from build123d import *

# Parameters (mm, degrees)
BASE_PLATE_SKETCH_R    = 15
BASE_PLATE_DEPTH       = 10
CENTRE_COLUMN_SKETCH_R = 15
CENTRE_COLUMN_DEPTH    = 50
TOP_PLATE_SKETCH_R     = 15
TOP_PLATE_DEPTH        = 10
OCTAGON_BOSS_SKETCH_R  = 25
OCTAGON_BOSS_DEPTH     = 10
CROSS_HOLE_18_D        = 18


with BuildPart() as part:
    # Base Plate Sketch → Base Plate (new body)
    with BuildSketch(Plane(origin=(0, 0, 0), x_dir=(1, 0, 0), z_dir=(0, 1, 0))):
        with BuildLine():
            Line((-40, 50), (40, 50))
            ThreePointArc((40, 50), (47.071067812, 47.071067812), (50, 40))
            Line((50, 40), (50, -40))
            ThreePointArc((50, -40), (47.071067812, -47.071067812), (40, -50))
            Line((40, -50), (-40, -50))
            ThreePointArc((-40, -50), (-47.071067812, -47.071067812), (-50, -40))
            Line((-50, -40), (-50, 40))
            ThreePointArc((-50, 40), (-47.071067812, 47.071067812), (-40, 50))
        make_face()
        with Locations(Location((0, 0, 0), (0, 0, 270))):
            Circle(BASE_PLATE_SKETCH_R, mode=Mode.SUBTRACT)
    extrude(amount=BASE_PLATE_DEPTH)

    # Centre Column Sketch → Centre Column (add)
    with BuildSketch(Plane(origin=(0, 10, 0), x_dir=(1, 0, 0), z_dir=(0, 1, 0))):
        with BuildLine():
            Line((-15, 30), (15, 30))
            ThreePointArc((15, 30), (25.606601718, 25.606601718), (30, 15))
            Line((30, 15), (30, -15))
            ThreePointArc((30, -15), (25.606601718, -25.606601718), (15, -30))
            Line((15, -30), (-15, -30))
            ThreePointArc((-15, -30), (-25.606601718, -25.606601718), (-30, -15))
            Line((-30, -15), (-30, 15))
            ThreePointArc((-30, 15), (-25.606601718, 25.606601718), (-15, 30))
        make_face()
        with Locations(Location((0, 0, 0), (0, 0, 270))):
            Circle(CENTRE_COLUMN_SKETCH_R, mode=Mode.SUBTRACT)
    extrude(amount=CENTRE_COLUMN_DEPTH)

    # Top Plate Sketch → Top Plate (add)
    with BuildSketch(Plane(origin=(0, 60, 0), x_dir=(1, 0, 0), z_dir=(0, 1, 0))):
        with BuildLine():
            Line((-40, -50), (40, -50))
            ThreePointArc((40, -50), (47.071067812, -47.071067812), (50, -40))
            Line((50, -40), (50, 40))
            ThreePointArc((50, 40), (47.071067812, 47.071067812), (40, 50))
            Line((40, 50), (-40, 50))
            ThreePointArc((-40, 50), (-47.071067812, 47.071067812), (-50, 40))
            Line((-50, 40), (-50, -40))
            ThreePointArc((-50, -40), (-47.071067812, -47.071067812), (-40, -50))
        make_face()
        with Locations(Location((0, 0, 0), (0, 0, 270))):
            Circle(TOP_PLATE_SKETCH_R, mode=Mode.SUBTRACT)
    extrude(amount=TOP_PLATE_DEPTH)

    # Octagon Boss Sketch → Octagon Boss (add)
    with BuildSketch(Plane(origin=(0, 70, 0), x_dir=(1, 0, 0), z_dir=(0, 1, 0))):
        Polygon((34, -14.083261121), (34, 14.083261121), (14.083261121, 34), (-14.083261121, 34), (-34, 14.083261121), (-34, -14.083261121), (-14.083261121, -34), (14.083261121, -34), align=None)
        with Locations(Location((0, 0, 0), (0, 0, 270))):
            Circle(OCTAGON_BOSS_SKETCH_R, mode=Mode.SUBTRACT)
    extrude(amount=OCTAGON_BOSS_DEPTH)

    # Cross Hole Ø18 (through all)
    with Locations(Plane.XY.offset(30)):
        with Locations((0, 35)):
            Hole(CROSS_HOLE_18_D / 2)


solid = part.part
Could you check a few things on this model? Use its own coordinates, in mm. A direction names the side the tool comes from. Coordinates: 2 decimals unless noted, no trailing zeros. Order: outer loops, then holes, each group sorted by start corner. A loop starts at its lowest first (then second) coordinate and runs counter-clockwise, first axis right, second up.
Q1. Thinking about a two-plate mould opening in X: for faces 6 (the flat face through (7, 29, 30)), 7 (the cylindrical face through (-4.153, 27.015, 20.874)), 8 (the cylindrical face through (7.509, 74.93, 23.846)), 9 (the cylindrical face through (-25.49, 34.65, 25.72)), which applies, released by +X, released by -X, zero draft, split by the parting line, or undercut?
Q2. Suppose I cut it at D-D on x = 42.5. Please give me the cut outline in (y, z).
Q3. Suppose I cut it at A-A on x = 0. Give the number of separate pieces and of enclosed holes in the cut face, and give its area (3 significant figures).
Q4. Which directions (+Z, -Z, +X, -X, +Y, -Y) give clear straight access to the entire face, cutting with the end or side of a thin tool? Please do faces 1 (the flat face through (23.902, 74.93, 24.181)), 2 (the flat face through (24.181, 74.93, -23.902)), 3 (the cylindrical face through (-25.72, 34.65, -25.49)), 4 (the flat face through (-23.902, 74.93, -24.181)), 5 (the cylindrical face through (25.72, 34.65, 25.49)).
Q5. Suppose I cut it at B-B on z = 0. Please give me the cut outline in (x, y), and give its area (3 significant figures).
Q6. Will these pins go through, and if not, where does the flat tip stop? pin 1 (6 mm diameter, centred on y = 29, z = -28.5, fed in from -X); pin 2 (4 mm diameter, centred on x = 21, y = 36, fed in from +Z); pin 3 (15 mm diameter, centred on y = 47.5, z = 7.5, fed in from -X).
Q7. Please list where these lines run through material, in increasing order: L1, parallel to Y at x = -34, z = 38; L2, parallel to X at y = 76.5, z = 0; L3, parallel to Y at x = 0, z = -25.25.
Q8. Suppose I cut it at C-C on y = 35. Please give me the cut outline in (x, z), and give its area (3 significant figures).
Answer:
1. face 6: zero draft
1. face 7: undercut
1. face 8: undercut
1. face 9: released by -X
2. outline: (0, -49.68) - (10, -49.68) - (10, 49.68) - (0, 49.68) - close; (60, -49.68) - (70, -49.68) - (70, 49.68) - (60, 49.68) - close
3. separate pieces: 4
3. enclosed holes: 0
3. area: 2,540 mm2
4. face 1: +Z, +X, +Y
4. face 2: -Z, +X, +Y
4. face 3: -Z, -X
4. face 4: -Z, -X, +Y
4. face 5: +Z, +X
5. outline: (-50, 0) - (-15, 0) - (-15, 70) - (-25, 70) - (-25, 80) - (-34, 80) - (-34, 70) - (-50, 70) - (-50, 60) - (-30, 60) - (-30, 10) - (-50, 10) - close; (15, 0) - (50, 0) - (50, 10) - (30, 10) - (30, 60) - (50, 60) - (50, 70) - (34, 70) - (34, 80) - (25, 80) - (25, 70) - (15, 70) - close
5. area: 3,080 mm2
6. pin 1: stops at x = -25.71
6. pin 2: stops at z = 29.46
6. pin 3: stops at x = -30
7. L1: y = 0 to 10, 60 to 70
7. L2: x = -34 to -25, 25 to 34
7. L3: y = 0 to 26, 44 to 80
8. outline: (-30, -15) arc R15 ccw to (-15, -30) - (-9, -30) - (-9, -12) arc R15 cw to (-9, 12) - (-9, 30) - (-15, 30) arc R15 ccw to (-30, 15) - close; (9, -30) - (15, -30) arc R15 ccw to (30, -15) - (30, 15) arc R15 ccw to (15, 30) - (9, 30) - (9, 12) arc R15 cw to (9, -12) - close
8. area: 2,130 mm2
